Verification items for this drawing (mm, ordinates from the low corner). A direction names the side the tool comes from. Give positions to 0.01 mm unless a question says otherwise; leave off trailing zeros. Order: outer loops, then holes, each group sorted by start corner. A loop starts at its lowest first (then second) coordinate and runs counter-clockwise, first axis right, second up.
(1) Sectioned sample at C-C on z = 15.5. Record the cut outline in (x, y) (1 decimal).
(2) Sectioned sample at A-A on y = 37.5. Record the cut outline in (x, z), plus the area to 3 significant figures.
(3) Sectioned sample at D-D on z = 22. Record the cut outline in (x, y) (1 decimal).
(4) Gauge pin test, flat ends, axial feed: pin 1 (3 mm diameter, centred on y = 21.5, z = 23, fed in from -X); pin 2 (5 mm diameter, centred on y = 60.5, z = 6.5, fed in from +X); pin 3 (10 mm diameter, centred on x = 69, z = 43.5, fed in from -Y) (1 decimal). Record the tip position at first contact, or that the pin passes through.
(5) Sectioned sample at B-B on x = 73.5. Record the cut outline in (y, z) (1 decimal).
(6) Scan lines: L1, parallel to Z at x = 39.5, y = 86 (1 decimal); L2, parallel to X at y = 37, z = 30 (1 decimal); L3, parallel to Y at x = 40.5, z = 40 (1 decimal). Record each from-to range of solid material in increasing order.
(7) Access from +Z, -Z, +X, -X, +Y, -Y to the whole of each face (thin tool, end or side, straight path). Record for the marked faces 5, 6 and 7.
(8) Mould release check, pull along X, two halves, no side actions. Record for the marked faces 1, 2, 3 and 4: pulls with the +X half, pulls with the -X half, needs draft (parallel to the pull), parting line crosses it, or undercut.
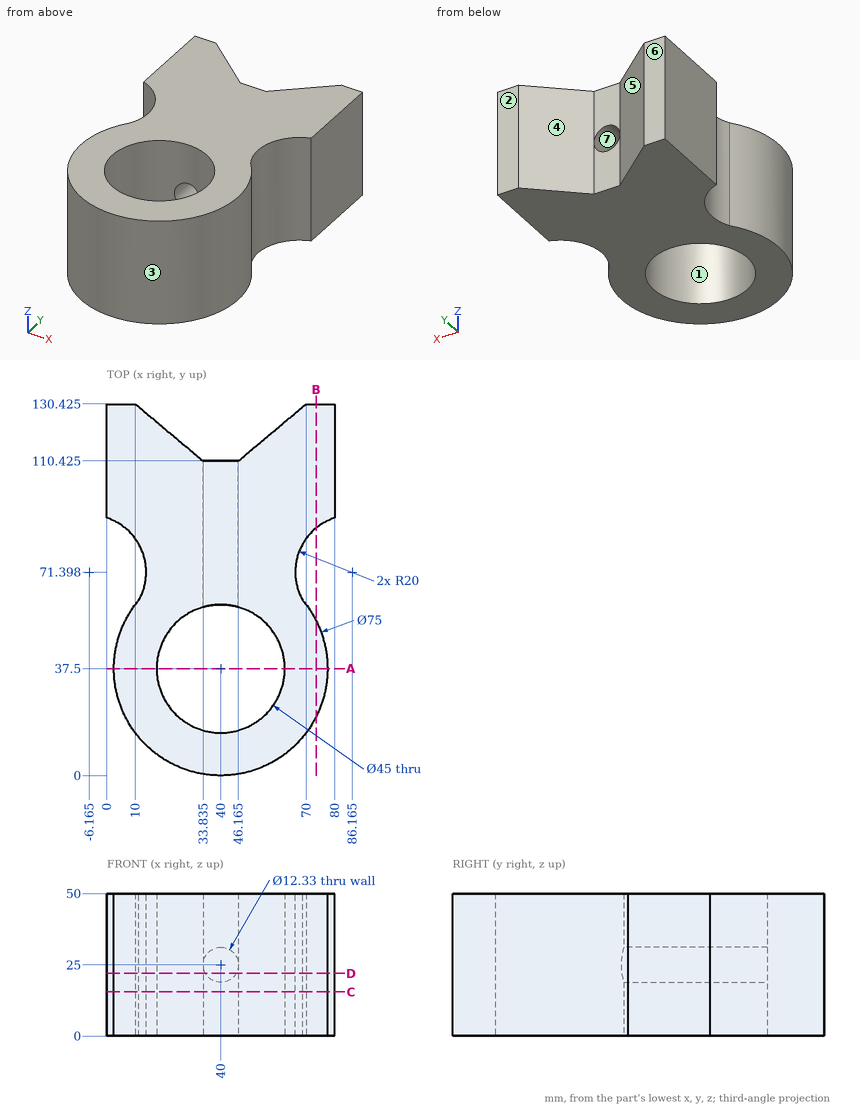
Ans:
1. outline: (0, 90.4) arc R20 cw to (11.3, 61.6) arc R37.5 ccw (long way) to (68.7, 61.6) arc R20 cw to (80, 90.4) - (80, 130.4) - (70, 130.4) - (46.2, 110.4) - (33.8, 110.4) - (10, 130.4) - (0, 130.4) - close; hole circle Ø45 at (40, 37.5)
2. outline: (2.5, 0) - (17.5, 0) - (17.5, 50) - (2.5, 50) - close; (62.5, 0) - (77.5, 0) - (77.5, 50) - (62.5, 50) - close
2. area: 1,500 mm2
3. outline: (0, 90.4) arc R20 cw to (11.3, 61.6) arc R37.5 ccw (long way) to (68.7, 61.6) arc R20 cw to (80, 90.4) - (80, 130.4) - (70, 130.4) - (46.2, 110.4) - (45.4, 110.4) - (45.4, 59.3) arc R22.5 cw (long way) to (34.6, 59.3) - (34.6, 110.4) - (33.8, 110.4) - (10, 130.4) - (0, 130.4) - close
4. pin 1: stops at x = 5.42
4. pin 2: stops at x = 71.4
4. pin 3: stops at y = 8.7
5. outline: (20.6, 0) - (54.4, 0) - (54.4, 50) - (20.6, 50) - close; (86.9, 0) - (130.4, 0) - (130.4, 50) - (86.9, 50) - close
6. L1: z = 0 to 18.9, 31.1 to 50
6. L2: x = 2.5 to 17.5, 62.5 to 77.5
6. L3: y = 0 to 15, 60 to 110.4
7. face 5: +Z, -Z, +Y
7. face 6: +Z, -Z, +X, -X, +Y
7. face 7: +Y
8. face 1: undercut
8. face 2: needs draft
8. face 3: parting line crosses it
8. face 4: undercut
